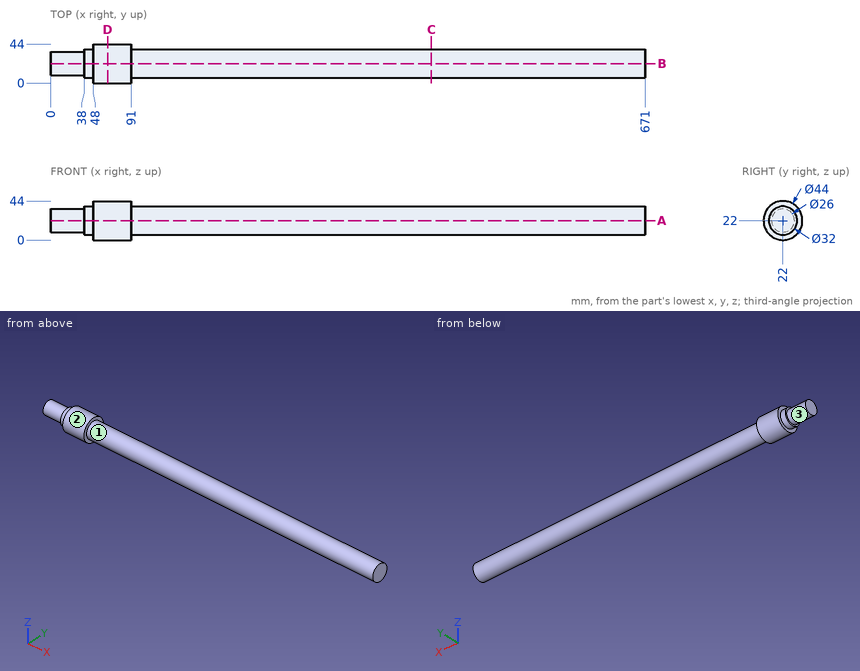
Design review of the part shown in the three views and the two pictorial views. Dimensions are in mm from the part's minimum x, y and z. A direction names the side the tool comes from. Coordinates: 2 decimals unless noted, no trailing zeros. Order: outer loops, then holes, each group sorted by start corner. A loop starts at its lowest first (then second) coordinate and runs counter-clockwise, first axis right, second up. Notation, with made-up numbers: (86.5, 88) - (104.5, 88) arc R23 cw to (104.5, 105) - close; hole circle Ø3 at (60, -10). An arc over 180 degrees is marked (long way). Answer as CSV lines item,"result". Start each with the question number.
1) To check wall thickness, follow line 1 along X through (y, z) = (17, 35.5); line 2 along X through (y, z) = (37, 37); line 3 along Z through (x, y) = (272, 14). State the ranges of each line that lie inside material, in increasing order. Write a range as [from, to].
2) Insertion check: P1, Ø1, axis at x = 137.5, z = 8.5, coming from the -Y side; P2, Ø8, axis at y = 10, z = 38.5, coming from the +X side; P3, Ø4, axis at x = 506.5, y = 21, coming from the -Z side. Each pin has a flat end and moves straight along its axis. Give the tip position at first contact, or say it passes through.
3) Machinability: for the marked faces 1, 2 and 3, which of the approach directions +Z, -Z, +X, -X, +Y, -Y give a long, thin tool a straight path to every point of the face, cutting with its end or side? Answer none if there is none.
4) Add section C-C (x = 429.5). State the section outline as (y, z) points.
5) Add section D-D (x = 64.5). State the section outline as (y, z) points.
6) Add section A-A (z = 22). State the section outline as (x, y) points, then the cut area to 3 significant figures.
Result:
1,line 1,"[38, 671]"
1,line 2,"[48, 91]"
1,line 3,"[8.14, 35.86]"
2,P1,"y = 12.67"
2,P2,"x = 91"
2,P3,"z = 6"
3,face 1,"+X"
3,face 2,"+X, -X"
3,face 3,"-X"
4,outline,"circle Ø32 at (22, 22)"
5,outline,"circle Ø44 at (22, 22)"
6,outline,"(0, 9) - (38, 9) - (38, 6) - (48, 6) - (48, 0) - (91, 0) - (91, 6) - (671, 6) - (671, 38) - (91, 38) - (91, 44) - (48, 44) - (48, 38) - (38, 38) - (38, 35) - (0, 35) - close"
6,area,"21,800 mm^2"
